The listing builds one solid part. Answer for the finished solid, in the listing's coordinates (mm). Face numbers are marked on the shaded views. Round coordinates to 2 decimals unless told otherwise and drop trailing zeros. Order: outer loops, then holes, each group sorted by start corner. A loop starts at its lowest first (then second) coordinate and runs counter-clockwise, first axis right, second up. Notation, with made-up numbers: (-8.75, 75.25) - (33.25, 75.25) arc R34 cw to (33.25, 108.25) - close; hole circle Ø11 at (-5, -18). An arc over 180 degrees is marked (long way). Write item = value, one per line.
from build123d import *

# Parameters (mm, degrees)
SKETCH1_R           = 3.5
SKETCH1_R_2         = 2.25
BOSS_EXTRUDE1_DEPTH = 7.5
CHAMFER1_SIZE       = 0.2


with BuildPart() as part:
    # Sketch1 → Boss-Extrude1 (new, symmetric)
    with BuildSketch(Plane.XY):
        Circle(SKETCH1_R)
        Circle(SKETCH1_R_2, mode=Mode.SUBTRACT)
    extrude(amount=BOSS_EXTRUDE1_DEPTH, both=True)

    # Chamfer1
    chamfer1_edges = [part.edges().sort_by_distance(p)[0] for p in [
        (-3.5, 0, -7.5),
        (-3.5, 0, 7.5),
        (-2.25, 0, -7.5),
        (-2.25, 0, 7.5),
    ]]
    chamfer(chamfer1_edges, length=CHAMFER1_SIZE)


solid = part.part
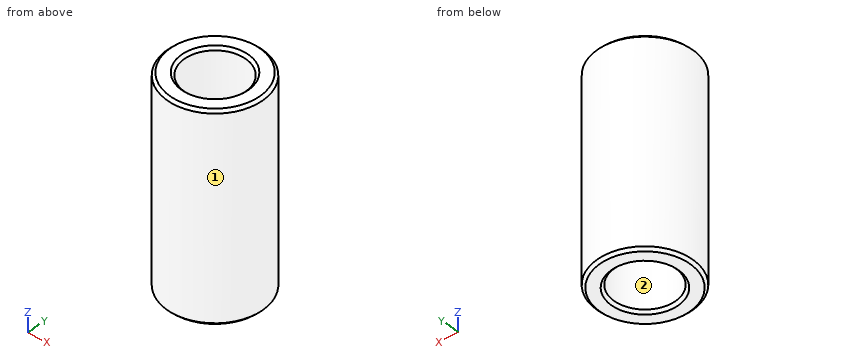
Q1. Find the intervals of material crossed by line 1 (Y direction, x = 0, z = 1.5); line 2 (Y direction, x = -2, z = -5.5); line 3 (X direction, y = -1.25, z = -0.5), in increasing order. Write a range as from..to.
Model answer:
line_1 = -3.5..-2.25, 2.25..3.5
line_2 = -2.87..-1.03, 1.03..2.87
line_3 = -3.27..-1.87, 1.87..3.27
Q2. Determine the mould class of the marked faces 1 and 2 for opening direction Y: released by +Y, released by -Y, zero draft, split by the parting line, or undercut.
Model answer:
face_1 = split by the parting line
face_2 = undercut
Q3. Section A-A on y = 0 is taken. Determine the outline of the cut face in (x, z), then the cut area to 3 significant figures.
Model answer:
outline = (-3.5, -7.3) - (-3.3, -7.5) - (-2.45, -7.5) - (-2.25, -7.3) - (-2.25, 7.3) - (-2.45, 7.5) - (-3.3, 7.5) - (-3.5, 7.3) - close; (2.25, -7.3) - (2.45, -7.5) - (3.3, -7.5) - (3.5, -7.3) - (3.5, 7.3) - (3.3, 7.5) - (2.45, 7.5) - (2.25, 7.3) - close
area = 37.3 mm^2
Q4. Section C-C on z = 4.5 is taken. Determine the outline of the cut face in (x, y).
Model answer:
outline = circle Ø7 at (0, 0); hole circle Ø4.5 at (0, 0)
